from build123d import *

# Parameters (mm, degrees)
SKETCH_1_R               = 16.5
EXTRUDE_1_DEPTH          = 12
SKETCH_2_R               = 3.75
CUT_EXTRUDE_1_DEPTH      = 4
EXTRUDE_START            = 2.5
EXTRUDE_2_DEPTH          = 2.5
PATTERN_CIRCULAR_1_COUNT = 4
SKETCH_4_R               = 2.25
SKETCH_4_R_2             = 2
CUT_EXTRUDE_2_DEPTH      = 4
SKETCH_5_W               = 5
SKETCH_5_H               = 5
CUT_EXTRUDE_3_DEPTH      = 2


with BuildPart() as part:
    # 草图1 → 凸台-拉伸1 (new body)
    with BuildSketch(Plane(origin=(0, 0, 0), x_dir=(0, 0, -1), z_dir=(1, 0, 0))):
        Circle(SKETCH_1_R)
    extrude(amount=EXTRUDE_1_DEPTH)

    # 草图2 → 切除-拉伸1 (cut)
    with BuildSketch(Plane.ZY):
        Circle(SKETCH_2_R)
    extrude(amount=-CUT_EXTRUDE_1_DEPTH, mode=Mode.SUBTRACT)

    # 草图3 → 凸台-拉伸2 (add)
    with BuildSketch(Plane.ZY.offset(EXTRUDE_START)):
        with BuildLine():
            Line((-3.639654287, -13.501149643), (-4.631065603, -15.836768338))
            ThreePointArc((-4.631065603, -15.836768338), (-6.44706362, -15.188330082), (-8.175009289, -14.332453493))
            Line((-8.175009289, -14.332453493), (-7.183597972, -11.996834798))
            Line((-7.183597972, -11.996834798), (-3.639654287, -13.501149643))
        make_face()
    extrude_2 = extrude(amount=-EXTRUDE_2_DEPTH)

    # 阵列(圆周)1: 凸台-拉伸2 ×4 about axis
    pattern_circular_1_axis = Axis((0, 0, 0), (1, 0, 0))
    for i in range(1, PATTERN_CIRCULAR_1_COUNT):
        add(extrude_2.rotate(pattern_circular_1_axis, i * 360 / PATTERN_CIRCULAR_1_COUNT))

    # 草图4 → 切除-拉伸2 (cut)
    with BuildSketch(Plane.ZY):
        with Locations((-1.282674839, 10.446548246)):
            Circle(SKETCH_4_R)
        with Locations((1.282674839, -10.446548246)):
            Circle(SKETCH_4_R_2)
    extrude(amount=-CUT_EXTRUDE_2_DEPTH, mode=Mode.SUBTRACT)

    # 草图5 → 切除-拉伸3 (cut)
    with BuildSketch(Plane(origin=(12, 0, 0), x_dir=(0, 0, -1), z_dir=(1, 0, 0))):
        Rectangle(SKETCH_5_W, SKETCH_5_H)
    extrude(amount=-CUT_EXTRUDE_3_DEPTH, mode=Mode.SUBTRACT)


solid = part.part
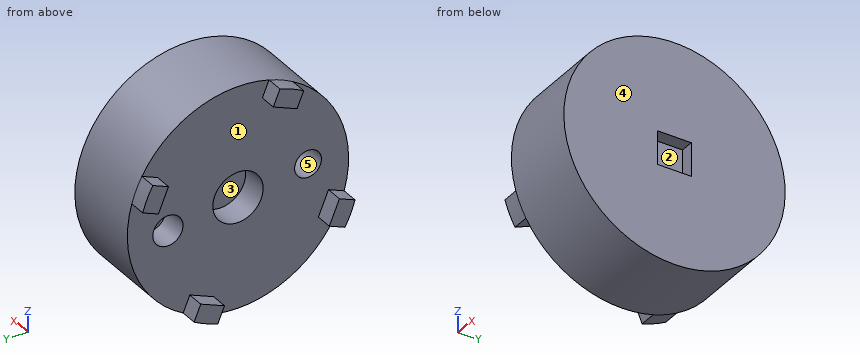
Can you work these out from the model? Positions are in its coordinate system, mm. Face numbers are marked on the shaded views. A direction names the side the tool comes from. Give positions to 0.01 mm unless a question says otherwise; leave off trailing zeros. Order: outer loops, then holes, each group sorted by start corner. A loop starts at its lowest first (then second) coordinate and runs counter-clockwise, first axis right, second up. Notation, with made-up numbers: M -39.75,25.5 L -27.75,25.5 A11 ccw -27.75,41.5 Z; hole C -29.75,27.5 d4. An arc over 180 degrees is marked long. One line per item, written item: value.
Item 1: For pin 1 (10 mm diameter, centred on y = -3.5, z = -5.5, fed in from -X); pin 2 (2 mm diameter, centred on x = 6.5, z = -8.5, fed in from -Y); pin 3 (4.5 mm diameter, centred on y = 0, z = 0, fed in from -X), each with a flat end and sliding along its axis, tell me the tip position at first contact or that it passes through.
Verdict:
pin 1: x = 0
pin 2: y = -14.7
pin 3: x = 4
Item 2: If we section it at C-C on z = -5.5: Write out the boundary of the cut face in (x, y), and give its area (3 significant figures).
Verdict:
outline: M -2.5,-15.56 L 12,-15.56 L 12,15.56 L 0,15.56 L 0,-12.71 L -2.5,-12.71 Z
area: 380 mm2
Item 3: Please list where these lines run through material, in increasing order: line 1 (X direction, y = -10.5, z = -12); line 2 (Y direction, x = 5.25, z = -0.5); line 3 (Z direction, x = 5.75, y = -13.5).
Verdict:
line 1: 0 to 12
line 2: -16.49 to 16.49
line 3: -9.49 to 9.49
Item 4: If we section it at B-B on y = 0: Write out the boundary of the cut face in (x, z), and give its area (3 significant figures).
Verdict:
outline: M 0,-16.5 L 12,-16.5 L 12,-2.5 L 10,-2.5 L 10,2.5 L 12,2.5 L 12,16.5 L 0,16.5 L 0,3.75 L 4,3.75 L 4,-3.75 L 0,-3.75 Z
area: 356 mm2
Item 5: If we section it at D-D on x = 8: Write out the boundary of the cut face in (y, z), and give its area (3 significant figures).
Verdict:
outline: C 0,0 d33
area: 855 mm2
Item 6: If we section it at A-A on x = -1.5: Write out the boundary of the cut face in (y, z) (3 decimals).
Verdict:
outline: M -15.837,-4.631 A16.5 ccw -14.332,-8.175 L -11.997,-7.184 L -13.501,-3.64 Z; M -8.175,14.332 L -7.184,11.997 L -3.64,13.501 L -4.631,15.837 A16.5 ccw Z; M 3.64,-13.501 L 4.631,-15.837 A16.5 ccw 8.175,-14.332 L 7.184,-11.997 Z; M 11.997,7.184 L 13.501,3.64 L 15.837,4.631 A16.5 ccw 14.332,8.175 Z
Item 7: If we mould it in two halves opening along Y, with no side actions, what happens to the marked faces 1, 2 and 3? For each: pulls with the +Y half, pulls with the -Y half, needs draft (parallel to the pull), parting line crosses it, or undercut.
Verdict:
face 1: needs draft
face 2: undercut
face 3: undercut
Item 8: For the marked faces 4 and 5, which set-ups out of +Z, -Z, +X, -X, +Y, -Y let a thin tool reach every point of the face, with its end or its side?
Verdict:
face 4: +Z, -Z, +X, +Y, -Y
face 5: -X
